Verification items for the finished model (mm, model axes). Face numbers are marked on the shaded views. A direction names the side the tool comes from. Give positions to 0.01 mm unless a question says otherwise; leave off trailing zeros. Write each loop counter-clockwise with the first axis right and the second up, starting at its lowest first coordinate (ties: lowest second). Pieces come first, ordered by that corner, then holes. Notation, with made-up numbers: (-18.5, 78.5) -> (-8.5, 78.5) arc R21 cw to (-8.5, 86.5) -> close; hole circle Ø10 at (-3.75, 56). An arc over 180 degrees is marked (long way). Answer as CSV lines item,"result". Start each with the question number.
1) Gauge pin test, flat ends, axial feed: pin 1 Ø8 at (x, z) = (-5, 28.5) entering from +Y; pin 2 Ø3 at (y, z) = (-2.5, 32.5) entering from -X; pin 3 Ø4 at (x, z) = (3, 37) entering from -Y. Record the tip position at first contact, or that the pin passes through.
2) Sectioned sample at A-A on y = 0. Record the cut outline in (x, z).
3) Sectioned sample at D-D on y = 7. Record the cut outline in (x, z).
4) Tool access check on the marked faces 1 and 2. Record the directions out of +Z, -Z, +X, -X, +Y, -Y that give a thin tool (end or side, any length) a straight path to the whole face; none if there is none.
5) Sectioned sample at B-B on z = 23. Record the cut outline in (x, y), and give its area (3 significant figures).
6) Material ranges on L1, parallel to Z at x = -6, y = 2.5; L2, parallel to X at y = 3.5, z = 28; L3, parallel to Y at x = 0.5, z = 47, recorded low to high.
7) Sectioned sample at C-C on x = -5.75. Record the cut outline in (y, z).
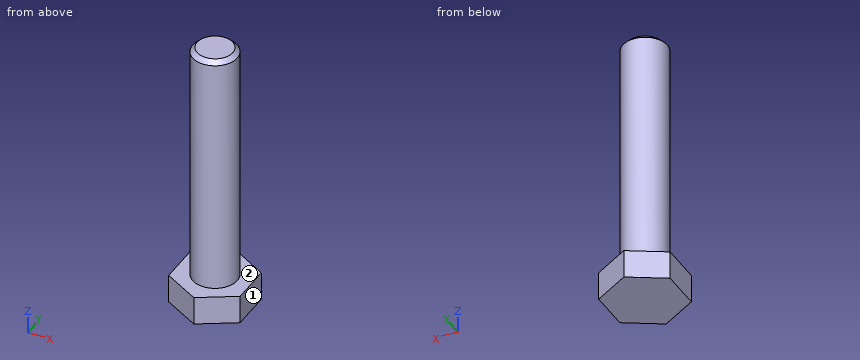
```python
from build123d import *

# Parameters (mm, degrees)
BOSS_EXTRUDE1_DEPTH = 6.4
SKETCH3_R           = 5
BOSS_EXTRUDE2_DEPTH = 55
CHAMFER1_SIZE       = 1


with BuildPart() as part:
    # Sketch1 → Boss-Extrude1 (new body)
    with BuildSketch(Plane.XY):
        Polygon((8, 4.618802154), (0, 9.237604307), (-8, 4.618802154), (-8, -4.618802154), (0, -9.237604307), (8, -4.618802154), align=None)
    extrude(amount=BOSS_EXTRUDE1_DEPTH)

    # Sketch3 → Boss-Extrude2 (add)
    with BuildSketch(Plane.XY.offset(6.4)):
        Circle(SKETCH3_R)
    extrude(amount=BOSS_EXTRUDE2_DEPTH)

    # Chamfer1
    chamfer1_edges = [part.edges().sort_by_distance(p)[0] for p in [
        (-5, 0, 61.4),
    ]]
    chamfer(chamfer1_edges, length=CHAMFER1_SIZE)


solid = part.part
```
Ans:
1,pin 1,"stops at y = 4.9"
1,pin 2,"stops at x = -4.9"
1,pin 3,"stops at y = -4.9"
2,outline,"(-8, 0) -> (8, 0) -> (8, 6.4) -> (5, 6.4) -> (5, 60.4) -> (4, 61.4) -> (-4, 61.4) -> (-5, 60.4) -> (-5, 6.4) -> (-8, 6.4) -> close"
3,outline,"(-3.88, 0) -> (3.88, 0) -> (3.88, 6.4) -> (-3.88, 6.4) -> close"
4,face 1,"+Z, -Z, +X, +Y, -Y"
4,face 2,"+Z"
5,outline,"circle Ø10 at (0, 0)"
5,area,"78.5 mm²"
6,L1,"z = 0 to 6.4"
6,L2,"x = -3.57 to 3.57"
6,L3,"y = -4.97 to 4.97"
7,outline,"(-5.92, 0) -> (5.92, 0) -> (5.92, 6.4) -> (-5.92, 6.4) -> close"
